```python
from build123d import *

# Parameters (mm, degrees)
SKETCH_1_W                = 125
SKETCH_1_H                = 156
EXTRUDE_1_DEPTH           = 12
SKETCH_2_W                = 55
SKETCH_2_H                = 36
CUT_EXTRUDE_1_DEPTH       = 101.669012114
SKETCH_3_W                = 70
SKETCH_3_H                = 35
CUT_EXTRUDE_2_DEPTH       = 3
HOLE_WIZARD_1_D           = 5.5
HOLE_WIZARD_1_CBORE_D     = 10
HOLE_WIZARD_1_CBORE_DEPTH = 5.7
HOLE_WIZARD_2_D           = 6.6
HOLE_WIZARD_2_CBORE_D     = 11
HOLE_WIZARD_2_CBORE_DEPTH = 6.8
CHAMFER_1_SIZE            = 2
FILLET_1_R                = 1


with BuildPart() as part:
    # 草图1 → 凸台-拉伸1 (new body)
    with BuildSketch(Plane.XY):
        Rectangle(SKETCH_1_W, SKETCH_1_H)
    extrude(amount=EXTRUDE_1_DEPTH)

    # 草图2 → 切除-拉伸1 (cut, through all)
    with BuildSketch(Plane.XY.offset(12)):
        with Locations((35, 60)):
            Rectangle(SKETCH_2_W, SKETCH_2_H)
    extrude(amount=-CUT_EXTRUDE_1_DEPTH, mode=Mode.SUBTRACT)

    # 草图3 → 切除-拉伸2 (cut)
    with BuildSketch(Plane(origin=(0, 0, 0), x_dir=(-1, 0, 0), z_dir=(0, 0, -1))):
        with Locations((27.5, 60.5)):
            Rectangle(SKETCH_3_W, SKETCH_3_H)
    extrude(amount=-CUT_EXTRUDE_2_DEPTH, mode=Mode.SUBTRACT)

    # 打孔尺寸(%根据)内六角圆柱头螺钉的类型1 (through all)
    with Locations(Plane(origin=(0, 0, 0), x_dir=(-1, 0, 0), z_dir=(0, 0, -1))):
        with Locations((-55, -72), (0, -72), (55, -72)):
            CounterBoreHole(HOLE_WIZARD_1_D / 2, HOLE_WIZARD_1_CBORE_D / 2, HOLE_WIZARD_1_CBORE_DEPTH)

    # 打孔尺寸(%根据)内六角圆柱头螺钉的类型2 (through all)
    with Locations(Plane(origin=(0, 0, 12), x_dir=(-1, 0, 0), z_dir=(0, 0, 1))):
        with Locations((2.5, -63), (27.5, -63), (52.5, -63)):
            CounterBoreHole(HOLE_WIZARD_2_D / 2, HOLE_WIZARD_2_CBORE_D / 2, HOLE_WIZARD_2_CBORE_DEPTH)

    # 倒角1
    chamfer_1_edges = [part.edges().sort_by_distance(p)[0] for p in [
        (62.5, 42, 6),
        (7.5, 78, 7.5),
        (62.5, -78, 6),
        (-62.5, -78, 6),
        (-62.5, 78, 7.5),
    ]]
    chamfer(chamfer_1_edges, length=CHAMFER_1_SIZE)

    # 圆角1
    fillet_1_edges = [part.edges().sort_by_distance(p)[0] for p in [
        (7.5, 42, 6),
    ]]
    fillet(fillet_1_edges, radius=FILLET_1_R)


solid = part.part
```
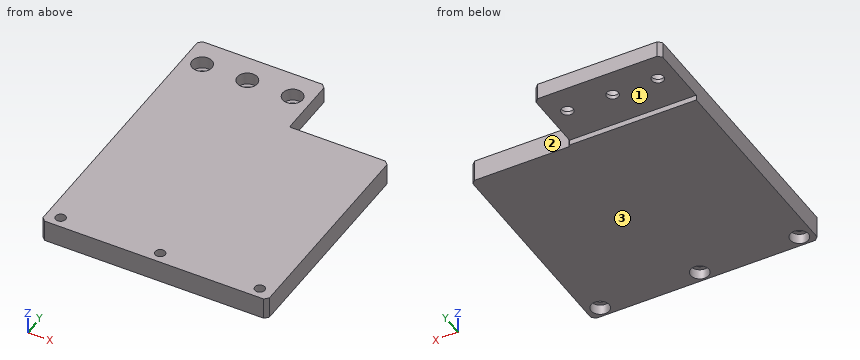
Part model, mm, in its own coordinate system. Face numbers are marked on the shaded views. A direction names the side the tool comes from. Round coordinates to 2 decimals unless told otherwise and drop trailing zeros. Loops run counter-clockwise (first coordinate to the right, second up) from the corner with the lowest first, then second, coordinate; pieces in that order, holes last. Notation, with made-up numbers: (-39, 3.25) -> (3, 3.25) arc R28 ccw to (3, 25.25) -> close; hole circle Ø4 at (54.25, -2). An arc over 180 degrees is marked (long way). Use a Markdown table: item, result.
1) Cut at C-C, the plane y = -72. List the corners of the cut face in (x, z).
The answers:
| item | result |
|---|---|
| outline | (-62.5, 0) -> (-60, 0) -> (-60, 5.7) -> (-57.75, 5.7) -> (-57.75, 12) -> (-62.5, 12) -> close; (-52.25, 5.7) -> (-50, 5.7) -> (-50, 0) -> (-5, 0) -> (-5, 5.7) -> (-2.75, 5.7) -> (-2.75, 12) -> (-52.25, 12) -> close; (2.75, 5.7) -> (5, 5.7) -> (5, 0) -> (50, 0) -> (50, 5.7) -> (52.25, 5.7) -> (52.25, 12) -> (2.75, 12) -> close; (57.75, 5.7) -> (60, 5.7) -> (60, 0) -> (62.5, 0) -> (62.5, 12) -> (57.75, 12) -> close |
2) Cut at A-A, the plane y = 63. List the corners of the cut face in (x, z).
The answers:
| item | result |
|---|---|
| outline | (-62.5, 3) -> (-55.8, 3) -> (-55.8, 5.2) -> (-58, 5.2) -> (-58, 12) -> (-62.5, 12) -> close; (-49.2, 3) -> (-30.8, 3) -> (-30.8, 5.2) -> (-33, 5.2) -> (-33, 12) -> (-47, 12) -> (-47, 5.2) -> (-49.2, 5.2) -> close; (-24.2, 3) -> (-5.8, 3) -> (-5.8, 5.2) -> (-8, 5.2) -> (-8, 12) -> (-22, 12) -> (-22, 5.2) -> (-24.2, 5.2) -> close; (0.8, 3) -> (7.5, 3) -> (7.5, 12) -> (3, 12) -> (3, 5.2) -> (0.8, 5.2) -> close |
3) Tool access for the marked faces 1, 2 and 3: list every direction of +Z, -Z, +X, -X, +Y, -Y with a clear straight run to the whole face (end or side of a thin tool).
The answers:
| item | result |
|---|---|
| face 1 | -Z, +X, -X, +Y |
| face 2 | +Z, -Z, +X, +Y |
| face 3 | -Z, +X, -X, +Y, -Y |
4) Cut at D-D, the plane x = -43.5. List the corners of the cut face in (y, z), and give its area (3 significant figures).
The answers:
| item | result |
|---|---|
| outline | (-78, 0) -> (43, 0) -> (43, 3) -> (78, 3) -> (78, 12) -> (-78, 12) -> close |
| area | 1,770 mm2 |
5) Drop flat-ended pins along their axis: pin 1 Ø6.5 at (x, y) = (-52.5, 63) entering from -Z; pin 2 Ø5 at (x, y) = (1, -72) entering from -Z; pin 3 Ø10.5 at (x, y) = (-2.5, 63) entering from -Z; pin 4 Ø3.5 at (x, z) = (27.5, 5.5) entering from +Y. Give the stop position or say it passes through.
The answers:
| item | result |
|---|---|
| pin 1 | passes through |
| pin 2 | stops at z = 5.7 |
| pin 3 | stops at z = 3 |
| pin 4 | stops at y = 42 |
6) Cut at B-B, the plane x = -27.5. List the corners of the cut face in (y, z), and give its area (3 significant figures).
The answers:
| item | result |
|---|---|
| outline | (-78, 0) -> (43, 0) -> (43, 3) -> (59.7, 3) -> (59.7, 5.2) -> (57.5, 5.2) -> (57.5, 12) -> (-78, 12) -> close; (66.3, 3) -> (78, 3) -> (78, 12) -> (68.5, 12) -> (68.5, 5.2) -> (66.3, 5.2) -> close |
| area | 1,680 mm2 |
7) Probe line 1 (X direction, y = 63, z = 3.6); line 2 (X direction, y = 63, z = 8); line 3 (Y direction, x = -2, z = 9). List the from-to ranges inside material, lowest first. Write a range as [from, to].
The answers:
| item | result |
|---|---|
| line 1 | x = [-62.5, -55.8], [-49.2, -30.8], [-24.2, -5.8], [0.8, 7.5] |
| line 2 | x = [-62.5, -58], [-47, -33], [-22, -8], [3, 7.5] |
| line 3 | y = [-78, -73.89], [-70.11, 57.52], [68.48, 78] |
